Source: CAD feature listing. Evaluate the final solid. Frame: model axes, mm. A direction names the side the tool comes from. Give positions to 0.01 mm unless a question says otherwise; leave off trailing zeros. Order: outer loops, then holes, each group sorted by start corner. A loop starts at its lowest first (then second) coordinate and runs counter-clockwise, first axis right, second up. Notation, with made-up numbers: (4.25, 83.5) -> (41.25, 83.5) arc R24 ccw to (41.25, 119.5) -> close; hole circle Ø1 at (77, -15). An arc over 180 degrees is marked (long way). Answer in a Markdown table with one row per item.
```python
from build123d import *

# Parameters (mm, degrees)
SKETCH1_R               = 24.5
BOSS_EXTRUDE1_DEPTH     = 2
SKETCH2_R               = 12
BOSS_EXTRUDE2_DEPTH     = 2.5
CUT_EXTRUDE1_DEPTH      = 35.939232962
CUT_EXTRUDE1_DEPTH_BACK = 2.5
SKETCH3_R               = 10.5
SKETCH4_R               = 2.5
CUT_EXTRUDE2_DEPTH      = 2.5
CHAMFER1_SIZE           = 0.5


with BuildPart() as part:
    # Sketch1 → Boss-Extrude1 (new body)
    with BuildSketch(Plane(origin=(0, 0, 0), x_dir=(0, 0, -1), z_dir=(1, 0, 0))):
        Circle(SKETCH1_R)
    extrude(amount=BOSS_EXTRUDE1_DEPTH)

    # Sketch2 → Boss-Extrude2 (add)
    with BuildSketch(Plane(origin=(2, 0, 0), x_dir=(0, 0, -1), z_dir=(1, 0, 0))):
        Circle(SKETCH2_R)
    extrude(amount=BOSS_EXTRUDE2_DEPTH)

    # Sketch3 → Cut-Extrude1 (cut, two sides: drawn at the far end of the back side and taken through both)
    with BuildSketch(Plane(origin=(4.5, 0, 0), x_dir=(0, 0, -1), z_dir=(1, 0, 0)).offset(-CUT_EXTRUDE1_DEPTH_BACK)):
        with Locations(Location((0, 0, 0), (0, 0, 180))):
            Circle(SKETCH3_R)
    extrude(amount=CUT_EXTRUDE1_DEPTH + CUT_EXTRUDE1_DEPTH_BACK, mode=Mode.SUBTRACT)

    # Sketch4 → Cut-Extrude2 (cut)
    with BuildSketch(Plane.ZY):
        with Locations((0, 20)):
            Circle(SKETCH4_R)
        with Locations((17.320508076, -10)):
            Circle(SKETCH4_R)
        with Locations((-17.320508076, -10)):
            Circle(SKETCH4_R)
    extrude(amount=-CUT_EXTRUDE2_DEPTH, mode=Mode.SUBTRACT)

    # Chamfer1
    chamfer1_edges = [part.edges().sort_by_distance(p)[0] for p in [
        (0, 0, 24.5),
        (4.5, 0, 12),
    ]]
    chamfer(chamfer1_edges, length=CHAMFER1_SIZE)


solid = part.part
```
(1) Section query C-C (x = 1.1). Return the cut outline in (y, z).
A:
| item | result |
|---|---|
| outline | circle Ø49 at (0, 0); hole circle Ø5 at (-10, -17.32); hole circle Ø5 at (-10, 17.32); hole circle Ø5 at (20, 0) |
(2) Pull-direction query (Y, two-part tool) for faces 3 (the cylindrical face through (0.99, 22.48, -0.33)), 4 (the flat face through (0, 0, 0)), 5 (the cylindrical face through (1.24, 20.66, -13.17)), 6 (the flat face through (2, 0, 0)); classes: +Y half, -Y half, draft (parallel to the pull), parting line (faces both ways), or undercut.
A:
| item | result |
|---|---|
| face 3 | undercut |
| face 4 | draft |
| face 5 | parting line |
| face 6 | undercut |
(3) Section query A-A (z = 0). Return the cut outline in (x, y), plus the area to 3 significant figures.
A:
| item | result |
|---|---|
| outline | (0, -24) -> (0.5, -24.5) -> (2, -24.5) -> (2, -12) -> (4, -12) -> (4.5, -11.5) -> (4.5, -10.5) -> (2, -10.5) -> (2, 10.5) -> (4.5, 10.5) -> (4.5, 11.5) -> (4, 12) -> (2, 12) -> (2, 17.5) -> (0, 17.5) -> close; (0, 22.5) -> (2, 22.5) -> (2, 24.5) -> (0.5, 24.5) -> (0, 24) -> close |
| area | 95.0 mm^2 |
(4) Ray query, probe 1 along Y at (x, z) = (1.2, 0); probe 2 along Y at (x, z) = (3.9, 0); probe 3 along X at (y, z) = (5.5, -22). Return the intervals inside material, ascending.
A:
| item | result |
|---|---|
| probe 1 | y = -24.5 to 17.5, 22.5 to 24.5 |
| probe 2 | y = -12 to -10.5, 10.5 to 12 |
| probe 3 | x = 0 to 2 |
(5) Section query B-B (y = 0). Return the cut outline in (x, z), plus the area to 3 significant figures.
A:
| item | result |
|---|---|
| outline | (0, -24) -> (0.5, -24.5) -> (2, -24.5) -> (2, -12) -> (4, -12) -> (4.5, -11.5) -> (4.5, -10.5) -> (2, -10.5) -> (2, 10.5) -> (4.5, 10.5) -> (4.5, 11.5) -> (4, 12) -> (2, 12) -> (2, 24.5) -> (0.5, 24.5) -> (0, 24) -> close |
| area | 105 mm^2 |
(6) First-contact query: pin 1 Ø6.5 at (y, z) = (-3.5, 3) entering from +X; pin 2 Ø4.5 at (y, z) = (20, 0) entering from -X; pin 3 Ø2 at (x, y) = (1.5, -6) entering from -Z. Flat tips, straight axial feed; report the tip coordinate or a pass-through.
A:
| item | result |
|---|---|
| pin 1 | stops at x = 2 |
| pin 2 | passes through |
| pin 3 | stops at z = -23.98 |
(7) Access query for faces 1 (the cylindrical face through (3.2, -3.2, 10)), 2 (the flat face through (4.5, -3.4, -10.2)). Directions: +Z, -Z, +X, -X, +Y, -Y. A direction counts if a zero-diameter tool reaches every point of the face in a straight line with its end or side. Return the directions, or none.
A:
| item | result |
|---|---|
| face 1 | +X |
| face 2 | +Z, -Z, +X, +Y, -Y |
